Part model, mm, in its own coordinate system. Face numbers are marked on the shaded views. A direction names the side the tool comes from. Give positions to 0.01 mm unless a question says otherwise; leave off trailing zeros. Write each loop counter-clockwise with the first axis right and the second up, starting at its lowest first coordinate (ties: lowest second). Pieces come first, ordered by that corner, then holes. Notation, with made-up numbers: M 2.5,26 L 11.5,26 A21 cw 11.5,65 Z; hole C -22,61.25 d10. An arc over 180 degrees is marked long. Use a Markdown table: item, result.
```python
from build123d import *

# Parameters (mm, degrees)
EXTRUDE_1_DEPTH        = 34
HOLE_WIZARD_M3_1_D     = 2.5
HOLE_WIZARD_M3_1_DEPTH = 7.5
HOLE_WIZARD_M3_1_TIP   = 0.751075774
CHAMFER_1_SIZE         = 1


with BuildPart() as part:
    # 草图1 → 凸台-拉伸1 (new body)
    with BuildSketch(Plane.XY):
        Polygon((-6, 0), (6, 0), (6, -5), (13.5, -5), (13.5, 5), (-13.5, 5), (-13.5, -5), (-6, -5), align=None)
    extrude(amount=EXTRUDE_1_DEPTH)

    # M3 螺纹孔1
    with Locations(Plane(origin=(0, 5, 0), x_dir=(1, 0, 0), z_dir=(0, 1, 0))):
        with Locations((-10, -9.5), (10, -9.5), (-10, -24.5), (10, -24.5)):
            Hole(HOLE_WIZARD_M3_1_D / 2, depth=HOLE_WIZARD_M3_1_DEPTH)
            with Locations((0, 0, -(HOLE_WIZARD_M3_1_DEPTH + HOLE_WIZARD_M3_1_TIP / 2))):  # 118° drill point
                Cone(0, HOLE_WIZARD_M3_1_D / 2, HOLE_WIZARD_M3_1_TIP, mode=Mode.SUBTRACT)

    # 倒角1
    chamfer_1_edges = [part.edges().sort_by_distance(p)[0] for p in [
        (-13.5, 5, 17),
        (13.5, 5, 17),
    ]]
    chamfer(chamfer_1_edges, length=CHAMFER_1_SIZE)


solid = part.part
```
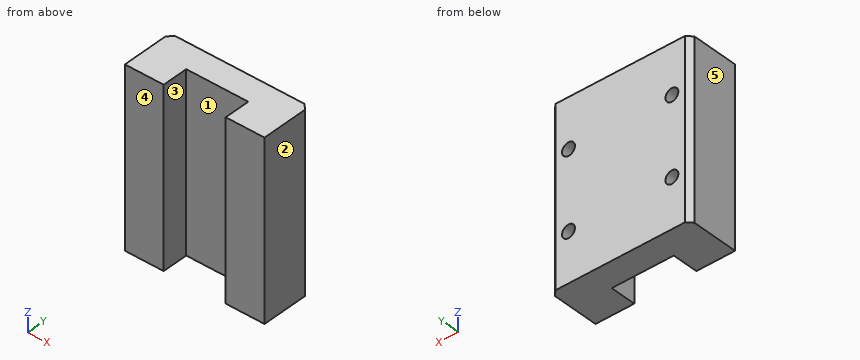
1. Drill centre lines: L1, parallel to Z at x = -10, y = 0; L2, parallel to X at y = 2.5, z = 9.5; L3, parallel to X at y = -0.75, z = 24.5. Where is each one in solid material? Low to high.
Findings below:
| item | result |
|---|---|
| L1 | 0 to 8.25, 10.75 to 23.25, 25.75 to 34 |
| L2 | -13.5 to -11.25, -8.75 to 8.75, 11.25 to 13.5 |
| L3 | -13.5 to -11.25, -8.75 to -6, 6 to 8.75, 11.25 to 13.5 |
2. Tool access for the marked faces 1 and 2: list every direction of +Z, -Z, +X, -X, +Y, -Y with a clear straight run to the whole face (end or side of a thin tool).
Findings below:
| item | result |
|---|---|
| face 1 | +Z, -Z, -Y |
| face 2 | +Z, -Z, +X, +Y, -Y |
3. Cut at C-C, the plane x = -2. Give the cut face in (y, z).
Findings below:
| item | result |
|---|---|
| outline | M 0,0 L 5,0 L 5,34 L 0,34 Z |
4. Drop flat-ended pins along their axis: P1, Ø2, axis at x = 10, z = 9.5, coming from the +Y side; P2, Ø1.5, axis at x = -4, z = 27.5, coming from the -Y side. Give the stop position or say it passes through.
Findings below:
| item | result |
|---|---|
| P1 | y = -2.65 |
| P2 | y = 0 |
5. Two-plate mould, pull along X, no slides. Class the marked faces 3, 4 and 5: released by +X, released by -X, zero draft, split by the parting line, or undercut.
Findings below:
| item | result |
|---|---|
| face 3 | undercut |
| face 4 | zero draft |
| face 5 | released by -X |
6. Cut at A-A, the plane y = 0.5. Give the cut face in (x, z).
Findings below:
| item | result |
|---|---|
| outline | M -13.5,0 L 13.5,0 L 13.5,34 L -13.5,34 Z; hole C -10,9.5 d2.5; hole C -10,24.5 d2.5; hole C 10,9.5 d2.5; hole C 10,24.5 d2.5 |
7. Cut at B-B, the plane z = 14.5. Give the cut face in (x, y).
Findings below:
| item | result |
|---|---|
| outline | M -13.5,-5 L -6,-5 L -6,0 L 6,0 L 6,-5 L 13.5,-5 L 13.5,4 L 12.5,5 L -12.5,5 L -13.5,4 Z |
